```python
from build123d import *

# Parameters (mm, degrees)
SKETCH1_W           = 212
SKETCH1_H           = 62
BOSS_EXTRUDE1_DEPTH = 26
SHELL1_T            = -7.5
SKETCH2_W           = 13
SKETCH2_H           = 2
CUT_EXTRUDE2_DEPTH  = 216.826319062
RIB1_REACH          = 115.459
SKETCH3_WALLS_W     = 6
SKETCH3_WALLS_H     = 275.918487568
SKETCH3_WALLS_H_2   = 275.934517232
BOSS_EXTRUDE2_REACH = 115.459


with BuildPart() as part:
    # Sketch1 → Boss-Extrude1 (new body)
    with BuildSketch(Plane(origin=(0, 0, 0), x_dir=(1, 0, 0), z_dir=(0, 1, 0))):
        Rectangle(SKETCH1_W, SKETCH1_H)
    extrude(amount=BOSS_EXTRUDE1_DEPTH)

    # Shell1
    shell1_openings = [part.faces().sort_by_distance(p)[0] for p in [
        (0, 0, 0),
    ]]
    offset(amount=SHELL1_T, openings=shell1_openings, kind=Kind.INTERSECTION)

    # Sketch2 → Cut-Extrude2 (cut, through all)
    with BuildSketch(Plane(origin=(106, 0, 0), x_dir=(0, 0, -1), z_dir=(1, 0, 0))):
        with Locations((24.5, 25)):
            Rectangle(SKETCH2_W, SKETCH2_H)
        with Locations((-24.5, 25)):
            Rectangle(SKETCH2_W, SKETCH2_H)
    extrude(amount=-CUT_EXTRUDE2_DEPTH, mode=Mode.SUBTRACT)

    # Sketch3 walls → Rib1 (add, up to next)
    with BuildSketch(Plane.XZ, mode=Mode.PRIVATE) as rib1_sk1:
        with Locations((45.5, 0)):
            Rectangle(SKETCH3_WALLS_W, SKETCH3_WALLS_H)
    rib1_tool1 = extrude(rib1_sk1.sketch, amount=-RIB1_REACH, mode=Mode.PRIVATE) - part.part
    # Sketch3 walls → Rib1 (add, up to next)
    with BuildSketch(Plane.XZ, mode=Mode.PRIVATE) as rib1_sk2:
        with Locations((-45.5, 0.008014832)):
            Rectangle(SKETCH3_WALLS_W, SKETCH3_WALLS_H_2)
    rib1_tool2 = extrude(rib1_sk2.sketch, amount=-RIB1_REACH, mode=Mode.PRIVATE) - part.part
    add(rib1_tool1.solids().sort_by_distance((45.5, 0, 0))[0])
    add(rib1_tool2.solids().sort_by_distance((-45.5, 0, 0.008014832))[0])

    # Sketch4 → Boss-Extrude2 (add, up to next)
    with BuildSketch(Plane.XZ, mode=Mode.PRIVATE) as boss_extrude2_sk1:
        Polygon((86.5, 23.5), (98.5, 11.5), (98.5, 23.5), align=None)
    boss_extrude2_tool1 = extrude(boss_extrude2_sk1.sketch, amount=-BOSS_EXTRUDE2_REACH, mode=Mode.PRIVATE) - part.part
    # Sketch4 → Boss-Extrude2 (add, up to next)
    with BuildSketch(Plane.XZ, mode=Mode.PRIVATE) as boss_extrude2_sk2:
        Polygon((-98.5, -11.5), (-86.5, -23.5), (-98.5, -23.5), align=None)
    boss_extrude2_tool2 = extrude(boss_extrude2_sk2.sketch, amount=-BOSS_EXTRUDE2_REACH, mode=Mode.PRIVATE) - part.part
    add(boss_extrude2_tool1.solids().sort_by_distance((94.5, 0, 19.5))[0])
    add(boss_extrude2_tool2.solids().sort_by_distance((-94.5, 0, -19.5))[0])


solid = part.part
```
The model under review builds one solid part; all positions refer to its coordinate system, in mm. A direction names the side the tool comes from. Give positions to 0.01 mm unless a question says otherwise; leave off trailing zeros. Write each loop counter-clockwise with the first axis right and the second up, starting at its lowest first coordinate (ties: lowest second). Pieces come first, ordered by that corner, then holes.
(1) Consider section A-A, the plane y = 15. Give the boundary of the cut face in (x, z), and give its area (3 significant figures).
(2) Consider section C-C, the plane x = -19. Give the boundary of the cut face in (y, z).
(3) Consider section D-D, the plane z = 27. Give the boundary of the cut face in (x, y), and give its area (3 significant figures).
(4) For P1, Ø0.6, axis at x = -2, y = 24.5, coming from the -Z side; P2, Ø1.5, axis at x = 35.5, z = 17.5, coming from the -Y side; P3, Ø4, axis at x = -22, z = 23.5, coming from the +Y side, all flat-tipped, find the tip position at first contact; note any pin that passes through.
(5) Tool access review of faces 5 (the flat face through (73, 9, -23.5)), 6 (the flat face through (1, 24, -24)), 7 (the flat face through (106, 13, 0)): name each direction out of +Z, -Z, +X, -X, +Y, -Y from which nothing blocks a thin tool from reaching the whole face with its end or side.
(6) Consider section B-B, the plane z = -9. Give the boundary of the cut face in (x, y), and give its area (3 significant figures).
(7) To check wall thickness, follow L1, parallel to X at y = 2.25, z = -6.5; L2, parallel to Z at x = -80, y = 6.75; L3, parallel to X at y = 11.5, z = 17.5. State the ranges of each line that lie inside material, in increasing order.
(8) The part is to be moulded in two halves that separate along Z. For faces 1 (the flat face through (42.5, 9, 0)), 2 (the flat face through (92, 9, 18)), 3 (the flat face through (-1, 12, 31)), 4 (the flat face through (1, 24, 25)), say which applies: released by +Z, released by -Z, zero draft, split by the parting line, or undercut.
Returned:
1. outline: (-106, -31) - (106, -31) - (106, 31) - (-106, 31) - close; hole (-98.5, -11.5) - (-86.5, -23.5) - (-48.5, -23.5) - (-48.5, 23.5) - (-98.5, 23.5) - close; hole (-42.5, -23.5) - (42.5, -23.5) - (42.5, 23.5) - (-42.5, 23.5) - close; hole (48.5, -23.5) - (98.5, -23.5) - (98.5, 11.5) - (86.5, 23.5) - (48.5, 23.5) - close
1. area: 4,590 mm2
2. outline: (0, -31) - (24, -31) - (24, -18) - (26, -18) - (26, 18) - (24, 18) - (24, 31) - (0, 31) - (0, 23.5) - (18.5, 23.5) - (18.5, -23.5) - (0, -23.5) - close
3. outline: (-106, 0) - (106, 0) - (106, 24) - (-106, 24) - close
3. area: 5,090 mm2
4. P1: stops at z = -18
4. P2: stops at y = 18.5
4. P3: stops at y = 24
5. face 5: -Y
5. face 6: -Z, +X, -X, +Y
5. face 7: +Z, -Z, +X, +Y, -Y
6. outline: (-106, 0) - (-98.5, 0) - (-98.5, 18.5) - (-48.5, 18.5) - (-48.5, 0) - (-42.5, 0) - (-42.5, 18.5) - (42.5, 18.5) - (42.5, 0) - (48.5, 0) - (48.5, 18.5) - (98.5, 18.5) - (98.5, 0) - (106, 0) - (106, 26) - (-106, 26) - close
6. area: 2,090 mm2
7. L1: x = -106 to -98.5, -48.5 to -42.5, 42.5 to 48.5, 98.5 to 106
7. L2: z = -31 to -23.5, 23.5 to 31
7. L3: x = -106 to -98.5, -48.5 to -42.5, 42.5 to 48.5, 92.5 to 106
8. face 1: undercut
8. face 2: undercut
8. face 3: released by +Z
8. face 4: zero draft
